```python
from build123d import *

# Parameters (mm, degrees)
SKETCH_1_W          = 12
SKETCH_1_H          = 95
EXTRUDE_1_DEPTH     = 50
CUT_EXTRUDE_1_REACH = 110.023
SKETCH_2_R          = 35.5
SKETCH_3_W          = 100
SKETCH_3_H          = 14
EXTRUDE_2_DEPTH     = 100
CHAMFER_1_SIZE      = 5


with BuildPart() as part:
    # 草图1 → 凸台-拉伸1 (new, symmetric)
    with BuildSketch(Plane.XY):
        with Locations((6, 47.5)):
            Rectangle(SKETCH_1_W, SKETCH_1_H)
    extrude(amount=EXTRUDE_1_DEPTH, both=True)

    # 草图2 → 切除-拉伸1 (cut, up to next)
    with BuildSketch(Plane(origin=(12, 0, 0), x_dir=(0, 0, -1), z_dir=(1, 0, 0)), mode=Mode.PRIVATE) as cut_extrude_1_sk1:
        with Locations(Location((0, 42, 0), (0, 0, 90))):
            Circle(SKETCH_2_R)
    cut_extrude_1_tool1 = extrude(cut_extrude_1_sk1.sketch, amount=-CUT_EXTRUDE_1_REACH, mode=Mode.PRIVATE) & part.part
    add(cut_extrude_1_tool1.solids().sort_by_distance((12, 42, 0))[0], mode=Mode.SUBTRACT)

    # 草图3 → 凸台-拉伸2 (add)
    with BuildSketch(Plane(origin=(12, 0, 0), x_dir=(0, 0, -1), z_dir=(1, 0, 0))):
        with Locations((0, 88)):
            Rectangle(SKETCH_3_W, SKETCH_3_H)
    extrude(amount=EXTRUDE_2_DEPTH)

    # 倒角1
    chamfer_1_edges = [part.edges().sort_by_distance(p)[0] for p in [
        (6, 0, 50),
        (6, 0, -50),
    ]]
    chamfer(chamfer_1_edges, length=CHAMFER_1_SIZE)


solid = part.part
```
For this review, take the finished solid that the model builds, in its own axes (mm). A direction names the side the tool comes from. Round coordinates to 2 decimals unless told otherwise and drop trailing zeros. Write each loop counter-clockwise with the first axis right and the second up, starting at its lowest first coordinate (ties: lowest second). Pieces come first, ordered by that corner, then holes. Notation, with made-up numbers: M 20,31.25 L 49,31.25 A5 cw 49,40.25 Z; hole C 38.25,56.25 d7. An arc over 180 degrees is marked long. One line per item, written item: value. Start each with the question number.
(1) We need section B-B (y = 42). Give the boundary of the cut face in (x, z).
(2) We need section D-D (z = -25). Give the boundary of the cut face in (x, y).
(3) Insertion check: pin 1 (10 mm diameter, centred on x = 37.5, z = 30.5, fed in from -Y); pin 2 (10 mm diameter, centred on x = 57, y = 74, fed in from -Z). Each pin has a flat end and moves straight along its axis. Give the tip position at first contact, or say it passes through.
(4) We need section A-A (z = 0). Give the boundary of the cut face in (x, y).
(5) We need section C-C (y = 9.5). Give the boundary of the cut face in (x, z), and give its area (3 significant figures).
(6) The part is to be moulded in two halves that separate along Z. For faces 3 (the cylindrical face through (6.08, 13.83, -21.6)), 4 (the flat face through (0, 79, 1)), 5 (the flat face through (6, 2, 47)), say which applies: released by +Z, released by -Z, zero draft, split by the parting line, or undercut.
(7) Machinability: for faces 1 (the flat face through (12, 13, 23)), 2 (the flat face through (35, 83, 50)), which of the approach directions +Z, -Z, +X, -X, +Y, -Y give a long, thin tool a straight path to every point of the face, cutting with its end or side? Answer none if there is none.
(8) Wall thickness on line 1 (Z direction, x = 6, y = 42); line 2 (Y direction, x = 32, z = 31); line 3 (Z direction, x = 7, y = 23): over which ranges is each line inside the solid? List them lowest first.
Result:
1. outline: M 0,-50 L 12,-50 L 12,-35.5 L 0,-35.5 Z; M 0,35.5 L 12,35.5 L 12,50 L 0,50 Z
2. outline: M 0,0 L 12,0 L 12,16.8 L 0,16.8 Z; M 0,67.2 L 12,67.2 L 12,81 L 112,81 L 112,95 L 0,95 Z
3. pin 1: y = 81
3. pin 2: through
4. outline: M 0,0 L 12,0 L 12,6.5 L 0,6.5 Z; M 0,77.5 L 12,77.5 L 12,81 L 112,81 L 112,95 L 0,95 Z
5. outline: M 0,-50 L 12,-50 L 12,-14.28 L 0,-14.28 Z; M 0,14.28 L 12,14.28 L 12,50 L 0,50 Z
5. area: 857 mm²
6. face 3: undercut
6. face 4: zero draft
6. face 5: released by +Z
7. face 1: +Z, -Z, +X, -Y
7. face 2: +Z, +X, -X, +Y, -Y
8. line 1: -50 to -35.5, 35.5 to 50
8. line 2: 81 to 95
8. line 3: -50 to -29.99, 29.99 to 50
